```python
from build123d import *

# Parameters (mm, degrees)
SKETCH1_W                                           = 210
SKETCH1_H                                           = 130
BOSS_EXTRUDE1_DEPTH                                 = 10
HOLE_SIZE_PER_SOCKET_HEAD_CAP_SCREW_TYP_D           = 6.6
HOLE_SIZE_PER_SOCKET_HEAD_CAP_SCREW_TYP_CBORE_D     = 11
HOLE_SIZE_PER_SOCKET_HEAD_CAP_SCREW_TYP_CBORE_DEPTH = 6.8
HOLE_SIZE_PER_SOCKET_HEAD_CAP_SCREW_2_D             = 5.5
HOLE_SIZE_PER_SOCKET_HEAD_CAP_SCREW_2_CBORE_D       = 10
HOLE_SIZE_PER_SOCKET_HEAD_CAP_SCREW_2_CBORE_DEPTH   = 5.7
CHAMFER1_SIZE                                       = 2


with BuildPart() as part:
    # Sketch1 → Boss-Extrude1 (new body)
    with BuildSketch(Plane.XY):
        Rectangle(SKETCH1_W, SKETCH1_H)
    extrude(amount=BOSS_EXTRUDE1_DEPTH)

    # Hole size _per socket head cap screw typ (through all)
    with Locations(Plane(origin=(-18, -17, 0), x_dir=(-1, 0, 0), z_dir=(0, 0, -1))):
        with Locations((0, 0), (-36, 0), (-36, 34), (0, 34)):
            CounterBoreHole(HOLE_SIZE_PER_SOCKET_HEAD_CAP_SCREW_TYP_D / 2, HOLE_SIZE_PER_SOCKET_HEAD_CAP_SCREW_TYP_CBORE_D / 2, HOLE_SIZE_PER_SOCKET_HEAD_CAP_SCREW_TYP_CBORE_DEPTH)

    # Hole size _per socket head cap screw 2 (through all)
    with Locations(Plane(origin=(-90, -55, 0), x_dir=(-1, 0, 0), z_dir=(0, 0, -1))):
        with Locations((0, 0), (0, 110), (-180, 110), (-180, 0)):
            CounterBoreHole(HOLE_SIZE_PER_SOCKET_HEAD_CAP_SCREW_2_D / 2, HOLE_SIZE_PER_SOCKET_HEAD_CAP_SCREW_2_CBORE_D / 2, HOLE_SIZE_PER_SOCKET_HEAD_CAP_SCREW_2_CBORE_DEPTH)

    # Chamfer1
    chamfer1_edges = [part.edges().sort_by_distance(p)[0] for p in [
        (105, -65, 5),
        (-105, -65, 5),
        (-105, 65, 5),
        (105, 65, 5),
    ]]
    chamfer(chamfer1_edges, length=CHAMFER1_SIZE)


solid = part.part
```
Verification items for the finished model (mm, model axes). A direction names the side the tool comes from. Coordinates: 2 decimals unless noted, no trailing zeros. Order: outer loops, then holes, each group sorted by start corner. A loop starts at its lowest first (then second) coordinate and runs counter-clockwise, first axis right, second up. Notation, with made-up numbers: (61, -39) -> (85, -39) arc R12 ccw to (85, -35) -> close; hole circle Ø9 at (-11.5, 40.25). An arc over 180 degrees is marked (long way). Put each result on its own line as item: value. Start each with the question number.
1) Release check for a two-part mould opening along X. For faces 3 (the flat face through (-1, -65, 5)), 4 (the flat face through (-105, -1, 5)), 5 (the cylindrical face through (12.92, -19.11, 3.35)) record: pulls with the +X half, pulls with the -X half, needs draft (parallel to the pull), parting line crosses it, or undercut.
2) Cross-section at B-B (y = 17). Enter the section's corners in (x, z).
3) Go/stop test with flat-tipped pins: pin 1 (7.5 mm diameter, centred on x = 18, y = 17, fed in from +Z); pin 2 (10.5 mm diameter, centred on x = -18, y = -17, fed in from -Z); pin 3 (8 mm diameter, centred on x = -90, y = 55, fed in from -Z). Record where each tip stops, or that it passes through.
4) Cross-section at A-A (x = -90). Enter the section's corners in (y, z), plus the area to 3 significant figures.
5) Material ranges on L1, parallel to Y at x = -18, z = 9.1; L2, parallel to X at y = -55.5, z = 7.25; L3, parallel to X at y = 59, z = 0.5, recorded low to high.
6) Tool access check on faces 1 (the cylindrical face through (89.642, -52.273, 7.88)), 2 (the flat face through (18, 13, 6.8)). Record the directions out of +Z, -Z, +X, -X, +Y, -Y that give a thin tool (end or side, any length) a straight path to the whole face; none if there is none.
Geometry check:
1. face 3: needs draft
1. face 4: pulls with the -X half
1. face 5: undercut
2. outline: (-105, 0) -> (-23.5, 0) -> (-23.5, 6.8) -> (-21.3, 6.8) -> (-21.3, 10) -> (-105, 10) -> close; (-14.7, 6.8) -> (-12.5, 6.8) -> (-12.5, 0) -> (12.5, 0) -> (12.5, 6.8) -> (14.7, 6.8) -> (14.7, 10) -> (-14.7, 10) -> close; (21.3, 6.8) -> (23.5, 6.8) -> (23.5, 0) -> (105, 0) -> (105, 10) -> (21.3, 10) -> close
3. pin 1: stops at z = 10
3. pin 2: stops at z = 6.8
3. pin 3: stops at z = 5.7
4. outline: (-65, 0) -> (-60, 0) -> (-60, 5.7) -> (-57.75, 5.7) -> (-57.75, 10) -> (-65, 10) -> close; (-52.25, 5.7) -> (-50, 5.7) -> (-50, 0) -> (50, 0) -> (50, 5.7) -> (52.25, 5.7) -> (52.25, 10) -> (-52.25, 10) -> close; (57.75, 5.7) -> (60, 5.7) -> (60, 0) -> (65, 0) -> (65, 10) -> (57.75, 10) -> close
4. area: 1,140 mm^2
5. L1: y = -65 to -20.3, -13.7 to 13.7, 20.3 to 65
5. L2: x = -105 to -92.7, -87.3 to 87.3, 92.7 to 105
5. L3: x = -105 to -93, -87 to 87, 93 to 105
6. face 1: +Z, -Z
6. face 2: -Z
